Here's how the part is built. I have some questions about the finished solid (model axes, mm). A direction names the side the tool comes from. Round coordinates to 2 decimals unless told otherwise and drop trailing zeros.
```python
from build123d import *

# Parameters (mm, degrees)
WEB_START                    = 111
WEB_RECESS_SKETCH_R          = 100
WEB_RECESS_DEPTH             = 100
LIGHTENING_HOLES_SKETCH_R    = 18
LIGHTENING_HOLES_4X_36_DEPTH = 50
HUB_SKETCH_R                 = 25
HUB_50_DEPTH                 = 24
BORE_KEYWAY_SKETCH_R         = 12.5
BORE_KEYWAY_SKETCH_W         = 10.879881684
BORE_KEYWAY_SKETCH_H         = 6
BORE_25_WITH_KEYWAY_DEPTH    = 100


with BuildPart() as part:
    # Pulley Profile Sketch → Pulley Body 3-Groove (revolve)
    with BuildSketch(Plane.XY, mode=Mode.PRIVATE) as pulley_body_3_groove_sk:
        Polygon((-2.5, 107), (2.5, 107), (9.051464217, 125), (14.051464217, 125), (20.602928434, 107), (25.602928434, 107), (32.15439265, 125), (40.84560735, 125), (40.84560735, 12.5), (-37.15439265, 12.5), (-37.15439265, 125), (-32.15439265, 125), (-25.602928434, 107), (-20.602928434, 107), (-14.051464217, 125), (-9.051464217, 125), align=None)
    revolve(pulley_body_3_groove_sk.sketch.rotate(Axis((491.806779687, 0, 0), (-1, 0, 0)), 90), axis=Axis((491.806779687, 0, 0), (-1, 0, 0)))

    # Web Recess Sketch → Web Recess (cut)
    with BuildSketch(Plane(origin=(0, 0, 0), x_dir=(0, 0, -1), z_dir=(1, 0, 0)).offset(WEB_START)):
        Circle(WEB_RECESS_SKETCH_R)
    web_recess = extrude(amount=-WEB_RECESS_DEPTH, mode=Mode.SUBTRACT)

    # Web Recess Mirror: Web Recess across plane
    add(web_recess.mirror(Plane(origin=(0, 0, 0), x_dir=(0, 0, 1), z_dir=(1, 0, 0))), mode=Mode.SUBTRACT)

    # Lightening Holes Sketch → Lightening Holes 4xØ36 (cut, symmetric)
    with BuildSketch(Plane(origin=(0, 0, 0), x_dir=(0, 0, -1), z_dir=(1, 0, 0))):
        with Locations((62.5, 0)):
            Circle(LIGHTENING_HOLES_SKETCH_R)
        with Locations((0, -62.5)):
            Circle(LIGHTENING_HOLES_SKETCH_R)
        with Locations((-62.5, 0)):
            Circle(LIGHTENING_HOLES_SKETCH_R)
        with Locations((0, 62.5)):
            Circle(LIGHTENING_HOLES_SKETCH_R)
    extrude(amount=LIGHTENING_HOLES_4X_36_DEPTH, both=True, mode=Mode.SUBTRACT)

    # Hub Sketch → Hub Ø50 (add, symmetric)
    with BuildSketch(Plane(origin=(0, 0, 0), x_dir=(0, 0, -1), z_dir=(1, 0, 0))):
        with Locations(Location((0, 0, 0), (0, 0, 180))):
            Circle(HUB_SKETCH_R)
    extrude(amount=HUB_50_DEPTH, both=True)

    # Bore Keyway Sketch → Bore Ø25 with Keyway (cut, symmetric)
    with BuildSketch(Plane(origin=(0, 0, 0), x_dir=(0, 0, -1), z_dir=(1, 0, 0))):
        Circle(BORE_KEYWAY_SKETCH_R)
        with Locations((10.060059158, 0.316113857)):
            Rectangle(BORE_KEYWAY_SKETCH_W, BORE_KEYWAY_SKETCH_H)
    extrude(amount=BORE_25_WITH_KEYWAY_DEPTH, both=True, mode=Mode.SUBTRACT)


solid = part.part
```
1) I'm going to push flat-ended pins straight in: pin 1 (6 mm diameter, centred on x = 33, z = -80.5, fed in from -Y); pin 2 (12 mm diameter, centred on x = 32.5, z = 57.5, fed in from -Y); pin 3 (6 mm diameter, centred on x = 31, z = -35.5, fed in from -Y). Where does each tip first touch, or does it pass through?
2) For faces 1 (the flat face through (-11, -21, -21)), 2 (the conical face through (-20.193, 105.555, 23.44)), 3 (the flat face through (11, -21, -21)), which set-ups out of +Z, -Z, +X, -X, +Y, -Y let a thin tool reach every point of the face, with its end or its side?
3) If we section it at A-A (z = 0): Give the number of separate pieces and of enclosed holes in the cut face, plus the area to 3 significant figures.
4) I need wall thicknesses on line 1 (Y direction, x = -10, z = -63.5); line 2 (X direction, y = 37.5, z = 27); line 3 (Y direction, x = -2, z = -14). Which ranges of each line are inside material? Lowest first, please.
5) We'd pull the mould along Z, two halves only. Please class faces 4 (the flat face through (-37.154, -84, -56)), 5 (the conical face through (2.91, 95.93, -49.89)), 6 (the cylindrical face through (0.3, 0.2, 12.5)): +Z half, -Z half, draft (parallel to the pull), parting line (faces both ways), or undercut.
Solutions:
1. pin 1: stops at y = -98.08
1. pin 2: stops at y = -113.9
1. pin 3: stops at y = -120.64
2. face 1: -X
2. face 2: none
2. face 3: +X
3. separate pieces: 4
3. enclosed holes: 0
3. area: 5,570 mm2
4. line 1: y = -107.67 to -17.97, 17.97 to 107.67
4. line 2: x = -11 to 11
4. line 3: y = -106.08 to -73.81, -51.19 to -2.68, 3.32 to 51.19, 73.81 to 106.08
5. face 4: draft
5. face 5: parting line
5. face 6: undercut
